```python
from build123d import *

# Parameters (mm, degrees)
BOSS_EXTRUDE1_DEPTH = 10
BOSS_EXTRUDE2_DEPTH = 20


with BuildPart() as part:
    # Sketch2 → Boss-Extrude1 (new body)
    with BuildSketch(Plane.XY):
        with BuildLine():
            Line((618.099915724, 106.517812479), (565.662842819, 90.936888582))
            ThreePointArc((565.662842819, 90.936888582), (576.256823377, 79.908186522), (577.354047602, 64.654964167))
            Line((577.354047602, 64.654964167), (623.40627245, 87.664511809))
            ThreePointArc((623.40627245, 87.664511809), (651.001261382, 85.576828369), (662.223491353, 60.280516566))
            Line((662.223491353, 60.280516566), (651.330966137, -29.057901231))
            ThreePointArc((651.330966137, -29.057901231), (629.656554116, -76.434863517), (584.606448191, -102.60440016))
            ThreePointArc((584.606448191, -102.60440016), (586.193547668, -107.242337985), (585.385803247, -112.077304476))
            ThreePointArc((585.385803247, -112.077304476), (631.589727703, -92.09112966), (654.31659075, -47.171874157))
            Line((654.31659075, -47.171874157), (667.921518172, 64.413150063))
            ThreePointArc((667.921518172, 64.413150063), (654.381801444, 98.92065746), (618.099915724, 106.517812479))
        make_face()
    extrude(amount=-BOSS_EXTRUDE1_DEPTH)

    # Sketch3 → Boss-Extrude2 (add)
    with BuildSketch(Plane.XY.offset(5)):
        with BuildLine():
            Line((616.390948328, 112.269284503), (549.290441383, 92.331331557))
            ThreePointArc((549.290441383, 92.331331557), (533.654573144, 66.258847309), (558.265088008, 48.410111539))
            Line((558.265088008, 48.410111539), (626.088009426, 82.297176642))
            ThreePointArc((626.088009426, 82.297176642), (647.542544399, 80.674045809), (656.267596834, 61.006684914))
            Line((656.267596834, 61.006684914), (645.375071617, -28.331732883))
            ThreePointArc((645.375071617, -28.331732883), (622.332456349, -75.416562354), (575.086767417, -98.127532436))
            ThreePointArc((575.086767417, -98.127532436), (566.230106721, -108.302539786), (575.565314818, -118.040357973))
            ThreePointArc((575.565314818, -118.040357973), (631.883168962, -99.833110413), (660.27248527, -47.898042505))
            Line((660.27248527, -47.898042505), (673.877412692, 63.686981716))
            ThreePointArc((673.877412692, 63.686981716), (658.254662621, 103.503336404), (616.390948328, 112.269284503))
        make_face()
        with BuildLine():
            ThreePointArc((618.099915724, 106.517812479), (654.381801444, 98.92065746), (667.921518172, 64.413150063))
            Line((667.921518172, 64.413150063), (654.31659075, -47.171874157))
            ThreePointArc((654.31659075, -47.171874157), (631.589727703, -92.09112966), (585.385803247, -112.077304476))
            ThreePointArc((585.385803247, -112.077304476), (586.193547668, -107.242337985), (584.606448191, -102.60440016))
            ThreePointArc((584.606448191, -102.60440016), (629.656554116, -76.434863517), (651.330966137, -29.057901231))
            Line((651.330966137, -29.057901231), (662.223491353, 60.280516566))
            ThreePointArc((662.223491353, 60.280516566), (651.001261382, 85.576828369), (623.40627245, 87.664511809))
            Line((623.40627245, 87.664511809), (577.354047602, 64.654964167))
            ThreePointArc((577.354047602, 64.654964167), (576.256823377, 79.908186522), (565.662842819, 90.936888582))
            Line((565.662842819, 90.936888582), (618.099915724, 106.517812479))
        make_face(mode=Mode.SUBTRACT)
        with BuildLine():
            ThreePointArc((557.409748377, 55.861178182), (540.79693583, 69.052632206), (553.988389854, 85.665444753))
            ThreePointArc((553.988389854, 85.665444753), (570.601202401, 72.47399073), (557.409748377, 55.861178182))
        make_face(mode=Mode.SUBTRACT)
        with BuildLine():
            ThreePointArc((576.797446678, -113.029665722), (571.259842496, -108.632514381), (575.656993837, -103.094910198))
            ThreePointArc((575.656993837, -103.094910198), (581.19459802, -107.492061539), (576.797446678, -113.029665722))
        make_face(mode=Mode.SUBTRACT)
    extrude(amount=-BOSS_EXTRUDE2_DEPTH)


solid = part.part
```
Design review of the part built by this model. Coordinates are the model's own, in mm. A direction names the side the tool comes from. Coordinates: 2 decimals unless noted, no trailing zeros. Order: outer loops, then holes, each group sorted by start corner. A loop starts at its lowest first (then second) coordinate and runs counter-clockwise, first axis right, second up.
1) Wall thickness on line 1 along X through (y, z) = (69, -5.5); line 2 along Y through (x, z) = (577.5, -0.25); line 3 along X through (y, z) = (76, -1): over which ranges is each line inside the solid? List them lowest first.
2) Mouldability with a two-part tool opening along Y and no side actions: class faces 5 (the flat face through (666.98, 7.11, -4.86)), 6 (the cylindrical face through (653.966, 99.267, 2.535)), 7 (the cylindrical face through (533.566, 66.718, -4.86)) as +Y half, -Y half, draft (parallel to the pull), parting line (faces both ways), or undercut.
3) Take a section at D-D, the plane y = -78.5. Give the boundary of the cut face in (x, z), and give its area (3 significant figures).
4) For faces 1 (the flat face through (661.214, 9.402, -12.465)), 2 (the flat face through (661.214, 9.402, 2.535)), 3 (the cylindrical face through (622.86, -74.89, -4.86)), 4 (the flat face through (591.702, 65.116, -4.86)), list the 3-axis set-ups (+Z, -Z, +X, -X, +Y, -Y) from which the entire face can be reached by the end or side of a thin tool; tool diameter is ignored.
5) Take a section at A-A, the plane z = -2.75. Give the boundary of the cut face in (x, y), and give its area (3 significant figures).
6) Take a section at C-C, the plane x = 612.5. Give the boundary of the cut face in (y, z), and give its area (3 significant figures).
7) Clearance check with flat-ended pins moving along their axes: pin 1 (1.5 mm diameter, centred on y = -22, z = -6.5, fed in from +X); pin 2 (1.5 mm diameter, centred on y = -41, z = -1, fed in from +X); pin 3 (10 mm diameter, centred on y = -71, z = -9, fed in from -X). State where each tip first meets the part, or that it passes through.
8) Take a section at B-B, the plane x = 642.5. Give the boundary of the cut face in (y, z).
Returned:
1. line 1: x = 533.27 to 540.8, 570.6 to 599.47, 655.7 to 674.21
1. line 2: y = -118.15 to -112.9, -103.23 to -97.81, 58.02 to 100.71
1. line 3: x = 533.82 to 541.64, 569.76 to 613.48, 652.32 to 673.68
2. face 5: -Y half
2. face 6: undercut
2. face 7: parting line
3. outline: (619.05, -15) - (627.72, -15) - (627.72, -10) - (642.93, -10) - (642.93, -15) - (649.98, -15) - (649.98, 5) - (642.93, 5) - (642.93, 0) - (627.72, 0) - (627.72, 5) - (619.05, 5) - close
3. area: 466 mm2
4. face 1: -Z
4. face 2: +Z
4. face 3: +Z, -Z, -X
4. face 4: +Z, -Z
5. outline: (549.29, 92.33) arc R22.5 ccw to (558.27, 48.41) - (626.09, 82.3) arc R20.96 cw to (656.27, 61.01) - (645.38, -28.33) arc R80 cw to (575.09, -98.13) arc R10 ccw to (575.57, -118.04) arc R80 ccw to (660.27, -47.9) - (673.88, 63.69) arc R45 ccw to (616.39, 112.27) - close; hole circle Ø30 at (555.7, 70.76); hole circle Ø10 at (576.23, -108.06)
5. area: 8,740 mm2
6. outline: (-111.69, -15) - (-105.11, -15) - (-105.11, -10) - (-90.97, -10) - (-90.97, -15) - (-83.72, -15) - (-83.72, 5) - (-90.97, 5) - (-90.97, 0) - (-105.11, 0) - (-105.11, 5) - (-111.69, 5) - close; (75.51, -15) - (82.22, -15) - (82.22, -10) - (104.85, -10) - (104.85, -15) - (111.11, -15) - (111.11, 5) - (104.85, 5) - (104.85, 0) - (82.22, 0) - (82.22, 5) - (75.51, 5) - close
6. area: 904 mm2
7. pin 1: stops at x = 663.52
7. pin 2: stops at x = 661.2
7. pin 3: stops at x = 621.74
8. outline: (-89.21, -15) - (-79.16, -15) - (-79.16, -10) - (-57.87, -10) - (-57.87, -15) - (-41.93, -15) - (-41.93, 5) - (-57.87, 5) - (-57.87, 0) - (-79.16, 0) - (-79.16, 5) - (-89.21, 5) - close; (83.29, -15) - (89.57, -15) - (89.57, -10) - (105.8, -10) - (105.8, -15) - (112.13, -15) - (112.13, 5) - (105.8, 5) - (105.8, 0) - (89.57, 0) - (89.57, 5) - (83.29, 5) - close
